Check sheet for the modelled part. Datum: model origin and axes. Units: mm. A direction names the side the tool comes from. Give positions to 0.01 mm unless a question says otherwise; leave off trailing zeros. Order: outer loops, then holes, each group sorted by start corner. A loop starts at its lowest first (then second) coordinate and runs counter-clockwise, first axis right, second up.
```python
from build123d import *

# Parameters (mm, degrees)
CUT_EXTRUDE1_DEPTH = 1.5


with BuildPart() as part:
    # Sketch1 → Revolve1 (revolve)
    with BuildSketch(Plane.XY, mode=Mode.PRIVATE) as revolve1_sk:
        Polygon((-3, 0), (-3, 2.383333333), (-2.633333333, 2.75), (0, 2.75), (0, 1.5), (11.6928325, 1.5), (12, 1.1928325), (12, 0), align=None)
    revolve(revolve1_sk.sketch.rotate(Axis((12, 0, 0), (-1, 0, 0)), 270), axis=Axis((12, 0, 0), (-1, 0, 0)))

    # Sketch2 → Cut-Revolve1 (revolve, cut)
    with BuildSketch(Plane.XY, mode=Mode.PRIVATE) as cut_revolve1_sk:
        Polygon((-3, 0), (-3, 1.25), (-1.5, 1.25), (-1.165063509, 0), align=None)
    revolve(cut_revolve1_sk.sketch.rotate(Axis((-1.165063509, 0, 0), (-1, 0, 0)), 270), axis=Axis((-1.165063509, 0, 0), (-1, 0, 0)), mode=Mode.SUBTRACT)

    # Sketch3 → Cut-Extrude1 (cut)
    with BuildSketch(Plane(origin=(-3, 0, 0), x_dir=(0, 0, -1), z_dir=(1, 0, 0))):
        Polygon((-1.25, 0.721687836), (-1.25, -0.721687836), (0, -1.443375673), (1.25, -0.721687836), (1.25, 0.721687836), (0, 1.443375673), align=None)
    extrude(amount=CUT_EXTRUDE1_DEPTH, mode=Mode.SUBTRACT)


solid = part.part
```
Q1. Draft check along Y on faces 4 (the cylindrical face through (-1.298, -2.685, -0.596)), 5 (the flat face through (0, -1.2, 1.2)), 6 (the flat face through (-2, 0, 1.25)). Enter one of: pulls with the +Y half, pulls with the -Y half, needs draft (parallel to the pull), parting line crosses it, or undercut.
Q2. Sectioned sample at A-A, the plane x = 5.75. Record the cut outline in (y, z), plus the area to 3 significant figures.
Q3. Tool access check on faces 1 (the flat face through (12, 0, 0)), 2 (the flat face through (-2.26, -1.088, -0.616)), 3 (the cylindrical face through (5.93, 0.45, 1.43)). Record the directions out of +Z, -Z, +X, -X, +Y, -Y that give a thin tool (end or side, any length) a straight path to the whole face; none if there is none.
Q4. Go/stop test with flat-tipped pins: P1, Ø2, axis at x = 3.5, z = -1.5, coming from the +Y side; P2, Ø3, axis at x = 3, z = 1, coming from the +Y side. Record where each tip stops, or that it passes through.
Q5. Material ranges on line 1 (X direction, y = -2.05, z = 0.1); line 2 (Y direction, x = -2, z = -1.1); line 3 (Z direction, x = 9.5, y = -0.1), recorded low to high.
Filled in:
1. face 4: parting line crosses it
1. face 5: needs draft
1. face 6: undercut
2. outline: circle Ø3 at (0, 0)
2. area: 7.07 mm2
3. face 1: +Z, -Z, +X, +Y, -Y
3. face 2: -X
3. face 3: +X
4. P1: stops at y = 1.41
4. P2: stops at y = 1.5
5. line 1: x = -3 to 0
5. line 2: y = -2.52 to -0.81, 0.81 to 2.52
5. line 3: z = -1.5 to 1.5
